Input: part model. Units: mm. Frame: model coordinates. Coordinates: 2 decimals unless noted, no trailing zeros. Loops run counter-clockwise (first coordinate to the right, second up) from the corner with the lowest first, then second, coordinate; pieces in that order, holes last.
Item 1: Ray query, line 1 along Y through (x, z) = (0, 1.45); line 2 along X through (y, z) = (-2.5, 0.2); line 3 along X through (y, z) = (-5.5, 0.55). Return the intervals inside material, ascending.
Item 2: Section B-B on y = -10.5. Return loops of the section in (x, z).
Item 3: Section A-A on z = 1. Return loops of the section in (x, y), and give its area (3 significant figures).
Item 4: Section C-C on x = -14.5. Return loops of the section in (y, z), and give its area (3 significant figures).
```python
from build123d import *

# Parameters (mm, degrees)
SKETCH1_R           = 3
BOSS_EXTRUDE1_DEPTH = 2


with BuildPart() as part:
    # Sketch1 → Boss-Extrude1 (new body)
    with BuildSketch(Plane.XY):
        with BuildLine():
            Line((-51.293623615, 5.521870404), (0, 9))
            ThreePointArc((0, 9), (9, 0), (0, -9))
            Line((0, -9), (-50.078661895, -12.395745198))
            ThreePointArc((-50.078661895, -12.395745198), (-60.273003894, -4.087005439), (-51.293623615, 5.521870404))
        make_face()
        with Locations((-51.293623615, -3.478129596)):
            Circle(SKETCH1_R, mode=Mode.SUBTRACT)
        Circle(SKETCH1_R, mode=Mode.SUBTRACT)
        with Locations((-25.646811807, -1.739064798)):
            Circle(SKETCH1_R, mode=Mode.SUBTRACT)
    extrude(amount=BOSS_EXTRUDE1_DEPTH)


solid = part.part
```
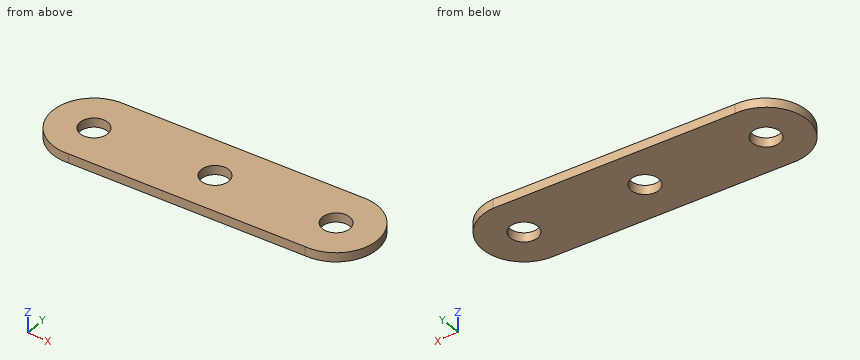
Results found:
1. line 1: y = -9 to -3, 3 to 9
1. line 2: x = -60.24 to -54.13, -48.46 to -28.55, -22.74 to -1.66, 1.66 to 8.65
1. line 3: x = -60.06 to -53.51, -49.08 to 7.12
2. outline: (-56.92, 0) - (-22.12, 0) - (-22.12, 2) - (-56.92, 2) - close
3. outline: (-51.29, 5.52) arc R9 ccw (long way) to (-50.08, -12.4) - (0, -9) arc R9 ccw to (0, 9) - close; hole circle Ø6 at (-51.29, -3.48); hole circle Ø6 at (-25.65, -1.74); hole circle Ø6 at (0, 0)
3. area: 1,090 mm2
4. outline: (-9.98, 0) - (8.02, 0) - (8.02, 2) - (-9.98, 2) - close
4. area: 36.0 mm2
